The figure shows three views and two pictorial views of one solid part (mm, origin at its lowest corner). Answer the questions. A direction names the side the tool comes from. Coordinates: 2 decimals unless noted, no trailing zeros. Loops run counter-clockwise (first coordinate to the right, second up) from the corner with the lowest first, then second, coordinate; pieces in that order, holes last. Notation, with made-up numbers: (40, 8.5) -> (54, 8.5) arc R20 cw to (54, 39.5) -> close; hole circle Ø9 at (62.25, -9.5). An arc over 180 degrees is marked (long way). Answer as a JSON object with one key per item and string values. Group by question number.
1) Section D-D, the plane y = 53 is taken. Give the vertices of the cut face in (x, z), plus the area to 3 significant figures.
2) Which of the six approach directions +Z, -Z, +X, -X, +Y, -Y give full straight-line access (tool end or side, diameter ignored) to the marked faces 1, 2, 3 and 4?
3) Determine the mould class of the marked faces 5, 6 and 7 for opening direction Z: released by +Z, released by -Z, zero draft, split by the parting line, or undercut.
4) Flat-ended cylindrical pins translate along their axes: P1, Ø1, axis at y = 54, z = 36.5, coming from the -X side; P2, Ø9, axis at x = 45, z = 24.5, coming from the +Y side; P3, Ø12, axis at x = 44, y = 29.5, coming from the -Z side; P4, Ø1.5, axis at y = 11.5, z = 11.5, coming from the +X side. Find the tip coordinate at first contact, or state that the pin passes through.
5) Section A-A, the plane x = 42 is taken. Give the vertices of the cut face in (y, z).
6) Section B-B, the plane y = 31 is taken. Give the vertices of the cut face in (x, z).
7) Consider probe 1 along X at (y, z) = (48, 44); probe 2 along Y at (x, z) = (40, 41); probe 3 along Y at (x, z) = (33, 15). Determine where each line is inside the solid, lowest interval first. Write a range as [from, to].
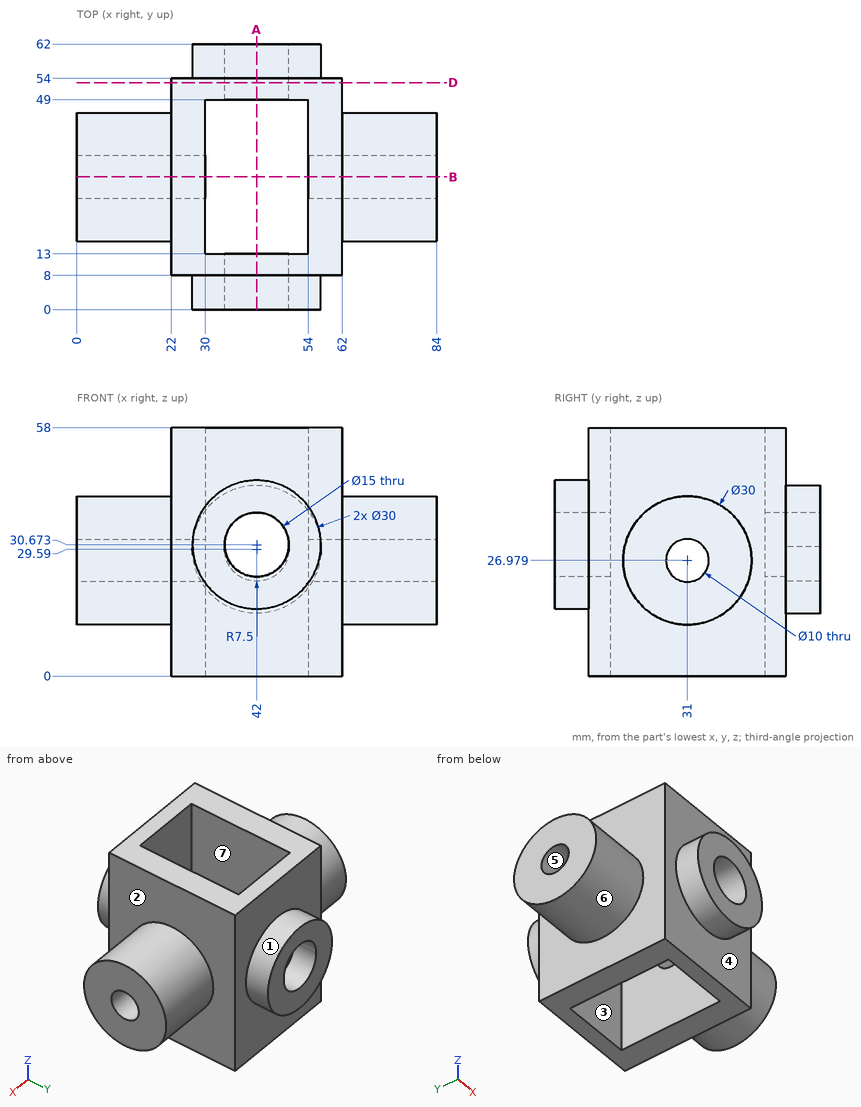
Determined:
{
 "1": {"outline": "(22, 0) -> (62, 0) -> (62, 58) -> (22, 58) -> close; hole circle Ø15 at (42, 30.67)", "area": "2,140 mm²"},
 "2": {"face 1": "+Y", "face 2": "+X", "face 3": "+Z, -Z", "face 4": "-Y"},
 "3": {"face 5": "undercut", "face 6": "split by the parting line", "face 7": "zero draft"},
 "4": {"P1": "x = 22", "P2": "y = 62", "P3": "through", "P4": "x = 62"},
 "5": {"outline": "(0, 15.67) -> (8, 15.67) -> (8, 0) -> (13, 0) -> (13, 23.17) -> (0, 23.17) -> close; (0, 38.17) -> (13, 38.17) -> (13, 58) -> (8, 58) -> (8, 45.67) -> (0, 45.67) -> close; (49, 0) -> (54, 0) -> (54, 14.59) -> (62, 14.59) -> (62, 22.09) -> (54, 22.09) -> (54, 23.17) -> (49, 23.17) -> close; (49, 38.17) -> (62, 38.17) -> (62, 44.59) -> (54, 44.59) -> (54, 58) -> (49, 58) -> close"},
 "6": {"outline": "(0, 11.98) -> (22, 11.98) -> (22, 0) -> (30, 0) -> (30, 21.98) -> (0, 21.98) -> close; (0, 31.98) -> (30, 31.98) -> (30, 58) -> (22, 58) -> (22, 41.98) -> (0, 41.98) -> close; (54, 0) -> (62, 0) -> (62, 11.98) -> (84, 11.98) -> (84, 21.98) -> (54, 21.98) -> close; (54, 31.98) -> (84, 31.98) -> (84, 41.98) -> (62, 41.98) -> (62, 58) -> (54, 58) -> close"},
 "7": {"probe 1": "[22, 30], [54, 62]", "probe 2": "[0, 13], [49, 62]", "probe 3": "[8, 13], [49, 54]"}
}
